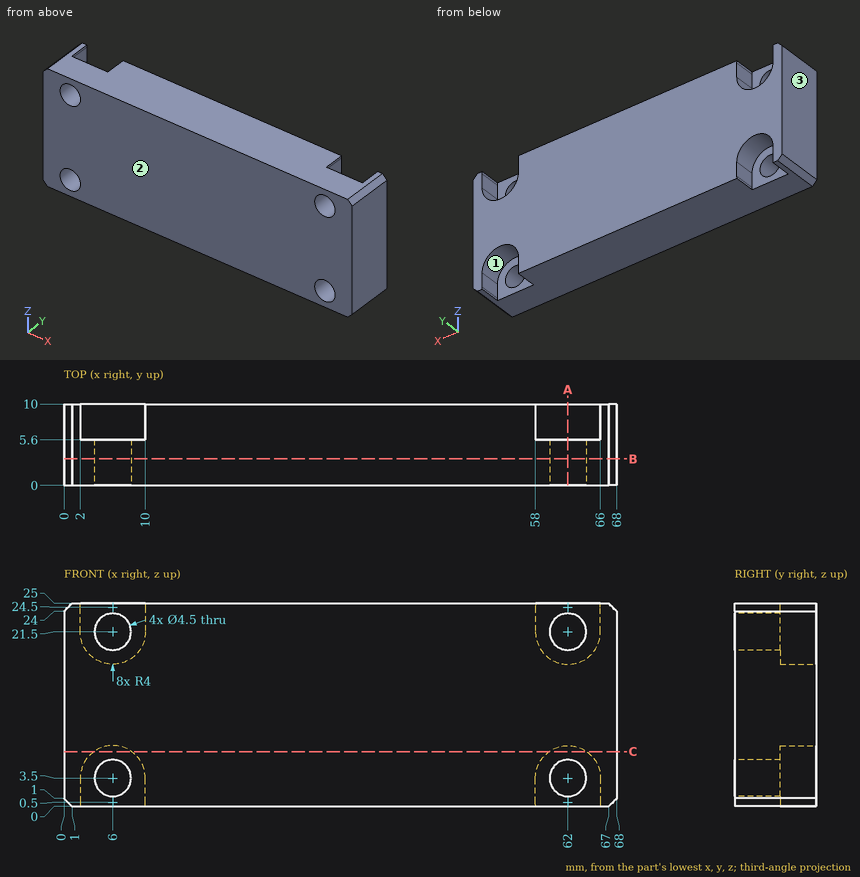
The figure shows three views and two pictorial views of one solid part (mm, origin at its lowest corner). Answer the questions. Give positions to 0.01 mm unless a question says otherwise; leave off trailing zeros. Write each loop counter-clockwise with the first axis right and the second up, starting at its lowest first coordinate (ties: lowest second). Pieces come first, ordered by that corner, then holes. Notation, with made-up numbers: (86, 79) -> (142, 79) arc R34 ccw to (142, 112) -> close; hole circle Ø11 at (68.5, 16). An arc over 180 degrees is marked (long way). Use one line per item in the form item = value.
1) Section C-C on z = 6.75 is taken. Write down the section's boundary in (x, y), plus the area to 3 significant figures.
Result:
outline = (0, 0) -> (68, 0) -> (68, 10) -> (64.33, 10) -> (64.33, 5.6) -> (59.67, 5.6) -> (59.67, 10) -> (8.33, 10) -> (8.33, 5.6) -> (3.67, 5.6) -> (3.67, 10) -> (0, 10) -> close
area = 639 mm²
2) Each of these flat-tipped pins is pushed along its axis until it touches: P1, Ø2, axis at x = 64, z = 19.5, coming from the +Y side; P2, Ø10, axis at x = 23, z = 8.5, coming from the -Y side; P3, Ø4, axis at x = 6, z = 3.5, coming from the +Y side. Where does it stop, or does it pass through?
Result:
P1 = 5.6
P2 = 0
P3 = through
3) Section B-B on y = 3.25 is taken. Write down the section's boundary in (x, z), plus the area to 3 significant figures.
Result:
outline = (0, 1) -> (1, 0) -> (67, 0) -> (68, 1) -> (68, 24) -> (67, 25) -> (1, 25) -> (0, 24) -> close; hole circle Ø4.5 at (6, 3.5); hole circle Ø4.5 at (6, 21.5); hole circle Ø4.5 at (62, 3.5); hole circle Ø4.5 at (62, 21.5)
area = 1,630 mm²
4) Straight lines are drawn through the part: probe 1 along Z at (x, y) = (6, 1.7); probe 2 along X at (y, z) = (1.8, 21.5). For each, find the intervals that lie inside material, in ascending order.
Result:
probe_1 = 0 to 1.25, 5.75 to 19.25, 23.75 to 25
probe_2 = 0 to 3.75, 8.25 to 59.75, 64.25 to 68
5) For a pull along X with two mould halves and no side action, classify the marked faces 1, 2 and 3 as +X half, -X half, draft (parallel to the pull), parting line (faces both ways), or undercut.
Result:
face_1 = undercut
face_2 = draft
face_3 = -X half
6) Section A-A on x = 62 is taken. Write down the section's boundary in (y, z).
Result:
outline = (0, 0) -> (5.6, 0) -> (5.6, 1.25) -> (0, 1.25) -> close; (0, 5.75) -> (5.6, 5.75) -> (5.6, 7.5) -> (10, 7.5) -> (10, 17.5) -> (5.6, 17.5) -> (5.6, 19.25) -> (0, 19.25) -> close; (0, 23.75) -> (5.6, 23.75) -> (5.6, 25) -> (0, 25) -> close
